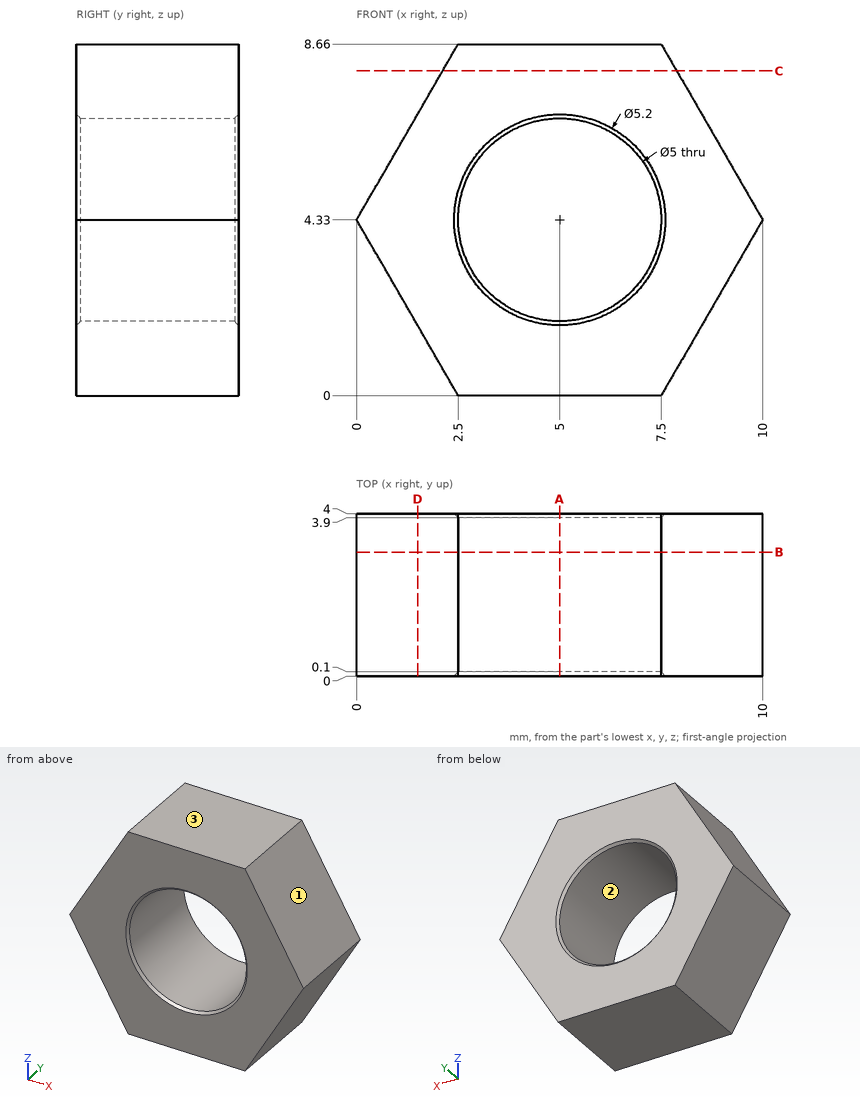
Design review of the part shown in the three views and the two pictorial views. Dimensions are in mm from the part's minimum x, y and z. Round coordinates to 2 decimals unless told otherwise and drop trailing zeros. Loops run counter-clockwise (first coordinate to the right, second up) from the corner with the lowest first, then second, coordinate; pieces in that order, holes last. Notation, with made-up numbers: (-28.5, -24) -> (-8.5, -24) arc R18 cw to (-8.5, -14) -> close; hole circle Ø3 at (59.5, -6.75). An arc over 180 degrees is marked (long way). Answer as CSV lines item,"result".
1) Add section B-B on y = 3.05. Write out the cut boundary in (x, z).
Geometry results:
outline,"(0, 4.33) -> (2.5, 0) -> (7.5, 0) -> (10, 4.33) -> (7.5, 8.66) -> (2.5, 8.66) -> close; hole circle Ø5 at (5, 4.33)"
2) To check wall thickness, follow line 1 along Z through (x, y) = (6, 1.85); line 2 along Z through (x, y) = (7, 2.7); line 3 along X through (y, z) = (2.7, 5). State the ranges of each line that lie inside material, in increasing order. Write a range as from..to.
Geometry results:
line 1,"z = 0..2.04, 6.62..8.66"
line 2,"z = 0..2.83, 5.83..8.66"
line 3,"x = 0.39..2.59, 7.41..9.61"
3) For P1, Ø2, axis at y = 2.5, z = 3, coming from the -X side, flat-tipped, find the tip position at first contact; note if it passes through.
Geometry results:
P1,"stops at x = 0.19"
4) Draft analysis for pull direction X (two halves, no side actions). For the marked faces 1, 2 and 3, state which applies: pulls with the +X half, pulls with the -X half, needs draft (parallel to the pull), parting line crosses it, or undercut.
Geometry results:
face 1,"pulls with the +X half"
face 2,"undercut"
face 3,"needs draft"
5) Add section A-A on x = 5. Write out the cut boundary in (y, z).
Geometry results:
outline,"(0, 0) -> (4, 0) -> (4, 1.73) -> (3.9, 1.83) -> (0.1, 1.83) -> (0, 1.73) -> close; (0, 6.93) -> (0.1, 6.83) -> (3.9, 6.83) -> (4, 6.93) -> (4, 8.66) -> (0, 8.66) -> close"
6) Add section C-C on z = 8. Write out the cut boundary in (x, y).
Geometry results:
outline,"(2.12, 0) -> (7.88, 0) -> (7.88, 4) -> (2.12, 4) -> close"
7) Add section D-D on x = 1.5. Write out the cut boundary in (y, z), plus the area to 3 significant figures.
Geometry results:
outline,"(0, 1.73) -> (4, 1.73) -> (4, 6.93) -> (0, 6.93) -> close"
area,"20.8 mm²"
